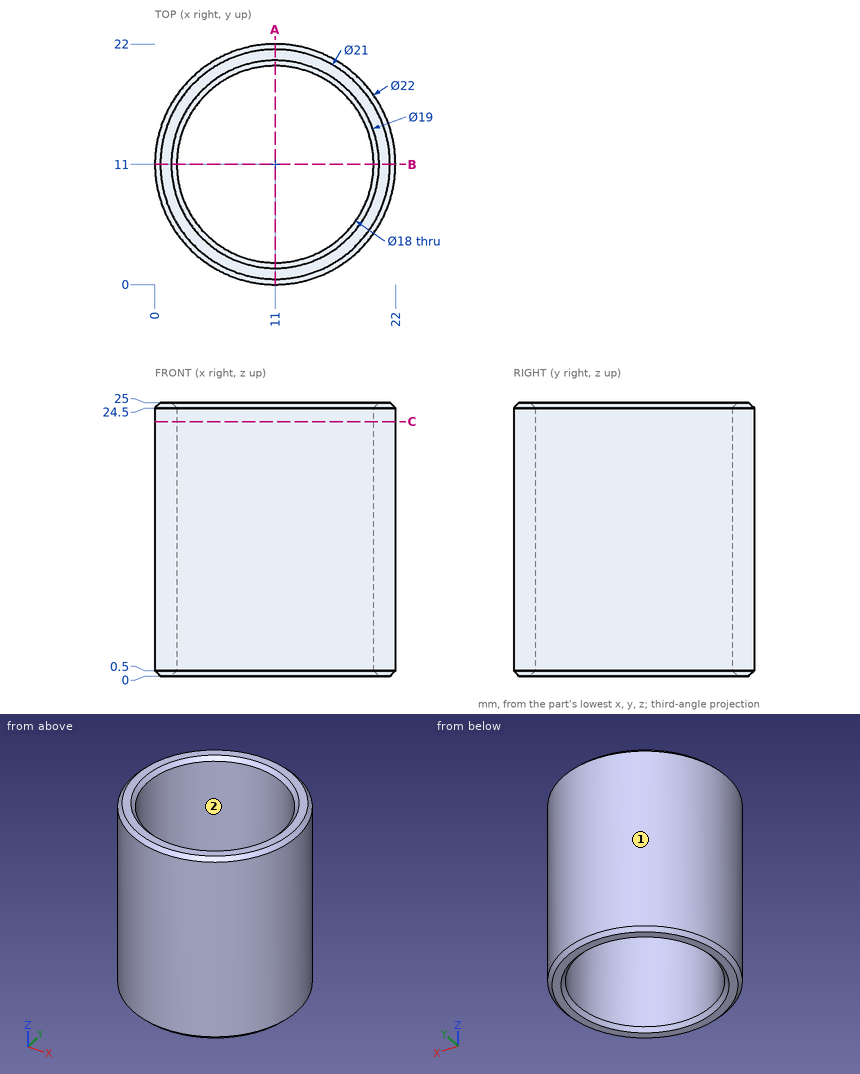
Input: dimensioned drawing with shaded views. Units: mm. Origin: part minimum x, y, z. Coordinates: 2 decimals unless noted, no trailing zeros. Order: outer loops, then holes, each group sorted by start corner. A loop starts at its lowest first (then second) coordinate and runs counter-clockwise, first axis right, second up.
(1) Material intervals for probe 1 along Y at (x, z) = (11, 15.75); probe 2 along X at (y, z) = (16, 7.75); probe 3 along X at (y, z) = (8.25, 5), sorted ascending.
(2) Section query C-C (z = 23.25). Return the cut outline in (x, y).
(3) Section query A-A (x = 11). Return the cut outline in (y, z).
(4) First-contact query: pin 1 (8 mm diameter, centred on x = 13, z = 22, fed in from -Y); pin 2 (2 mm diameter, centred on y = 16, z = 17.5, fed in from +X); pin 3 (1.5 mm diameter, centred on x = 19.5, z = 21.5, fed in from -Y); pin 4 (1 mm diameter, centred on x = 13.5, y = 2.5, fed in from -Z). Flat tips, straight axial feed; report the tip coordinate or a pass-through.
(5) Draft query along Y for the marked faces 1 and 2. Return one class per face: pulls with the +Y half, pulls with the -Y half, needs draft (parallel to the pull), parting line crosses it, or undercut.
Solution:
1. probe 1: y = 0 to 2, 20 to 22
1. probe 2: x = 1.2 to 3.52, 18.48 to 20.8
1. probe 3: x = 0.35 to 2.43, 19.57 to 21.65
2. outline: circle Ø22 at (11, 11); hole circle Ø18 at (11, 11)
3. outline: (0, 0.5) - (0.5, 0) - (1.5, 0) - (2, 0.5) - (2, 24.5) - (1.5, 25) - (0.5, 25) - (0, 24.5) - close; (20, 0.5) - (20.5, 0) - (21.5, 0) - (22, 0.5) - (22, 24.5) - (21.5, 25) - (20.5, 25) - (20, 24.5) - close
4. pin 1: stops at y = 0
4. pin 2: stops at x = 21.25
4. pin 3: stops at y = 3.19
4. pin 4: stops at z = 0.14
5. face 1: parting line crosses it
5. face 2: undercut
